Part model, mm, in its own coordinate system. A direction names the side the tool comes from. Give positions to 0.01 mm unless a question says otherwise; leave off trailing zeros. Write each loop counter-clockwise with the first axis right and the second up, starting at its lowest first coordinate (ties: lowest second). Pieces come first, ordered by that corner, then holes. Notation, with made-up numbers: (30, -10) - (57, -10) arc R38 ccw to (57, 28) - close; hole circle Ø3 at (50.25, -7.75). An arc over 180 degrees is marked (long way). Answer as a JSON object with one key per item and string values. Group by question number.
```python
from build123d import *

# Parameters (mm, degrees)
SKETCH_1_R          = 9.15
SKETCH_1_R_2        = 7.15
EXTRUDE_1_DEPTH     = 1
SKETCH_2_W          = 2
SKETCH_2_H          = 11.561648884
CUT_EXTRUDE_1_DEPTH = 13.978636292
EXTRUDE_START       = -1
SKETCH_3_R          = 0.4
EXTRUDE_2_DEPTH     = 1


with BuildPart() as part:
    # 草图1 → 拉伸1 (new body)
    with BuildSketch(Plane(origin=(0, 0, 0), x_dir=(0, 0, -1), z_dir=(1, 0, 0))):
        Circle(SKETCH_1_R)
        Circle(SKETCH_1_R_2, mode=Mode.SUBTRACT)
    extrude(amount=EXTRUDE_1_DEPTH)

    # 草图2 → 切除-拉伸1 (cut, through all)
    with BuildSketch(Plane(origin=(1, 0, 0), x_dir=(0, 0, -1), z_dir=(1, 0, 0))):
        with Locations((0, 5.780824442)):
            Rectangle(SKETCH_2_W, SKETCH_2_H)
    extrude(amount=-CUT_EXTRUDE_1_DEPTH, mode=Mode.SUBTRACT)

    # 草图3 → 拉伸2 (add)
    # profile 1 of 2: a face of its own
    with BuildSketch(Plane(origin=(1, 0, 0), x_dir=(0, 0, -1), z_dir=(1, 0, 0)).offset(EXTRUDE_START)):
        with BuildLine():
            Line((-1, 9.095191037), (-1, 10.12554219))
            Line((-1, 10.12554219), (-2.197020967, 10.125546621))
            ThreePointArc((-2.197020967, 10.125546621), (-2.744657845, 9.962265155), (-3.113455807, 9.525739038))
            Line((-3.113455807, 9.525739038), (-3.599741921, 8.412155378))
            ThreePointArc((-3.599741921, 8.412155378), (-2.325089431, 8.849658702), (-1, 9.095191037))
        make_face()
        with Locations((-2.0521454, 9.383212306)):
            Circle(SKETCH_3_R, mode=Mode.SUBTRACT)
    # profile 2 of 2: a face of its own
    with BuildSketch(Plane(origin=(1, 0, 0), x_dir=(0, 0, -1), z_dir=(1, 0, 0)).offset(EXTRUDE_START)):
        with BuildLine():
            Line((1, 9.095191037), (1, 10.12554219))
            Line((1, 10.12554219), (2.197020967, 10.125546621))
            ThreePointArc((2.197020967, 10.125546621), (2.744657845, 9.962265155), (3.113455807, 9.525739038))
            Line((3.113455807, 9.525739038), (3.599741921, 8.412155378))
            ThreePointArc((3.599741921, 8.412155378), (2.325089431, 8.849658702), (1, 9.095191037))
        make_face()
        with Locations(Location((2.0521454, 9.383212306, 0), (0, 0, 180))):
            Circle(SKETCH_3_R, mode=Mode.SUBTRACT)
    extrude(amount=EXTRUDE_2_DEPTH)


solid = part.part
```
1) Which spindle directions (+Z, -Z, +X, -X, +Y, -Y) get a long thin tool onto all of the face, cutting with end or side? Do faces 4 (the flat face through (0.5, 8.6, 1)), 5 (the flat face through (0, -7, 3)). Say none if no direction does.
2) Saw through at B-B (z = 6.25). List the corners of the cut face in (x, y).
3) Saw through at A-A (y = 0). List the corners of the cut face in (x, z).
4) Two-plate mould, pull along Z, no slides. Class faces 1 (the flat face through (0.49, 8.98, -3.35)), 2 (the cylindrical face through (0.493, -7.144, 0.3)), 3 (the cylindrical face through (0.493, -9.143, 0.351)): +Z half, -Z half, draft (parallel to the pull), parting line (faces both ways), or undercut.
5) Drop a flat-ended pin along its axis: P1, Ø5, axis at y = 6.5, z = 5.5, coming from the -X side. Give the stop position or say it passes through.
6) Saw through at D-D (z = 0). List the corners of the cut face in (x, y).
7) Drill centre lines: line 1 along Z through (x, y) = (0.7, -0.25); line 2 along Z through (x, y) = (0.7, 1.5); line 3 along Y through (x, z) = (0.85, -6.25). Where is each one in solid material? Low to high. Write a range as from..to.
8) Saw through at C-C (x = 0.5). List the corners of the cut face in (y, z), and give its area (3 significant figures).
Checks:
{
 "1": {"face 4": "+X, -X, +Y", "face 5": "+Z, -Z, -X, +Y, -Y"},
 "2": {"outline": "(0, -6.68) - (1, -6.68) - (1, -3.47) - (0, -3.47) - close; (0, 3.47) - (1, 3.47) - (1, 6.68) - (0, 6.68) - close"},
 "3": {"outline": "(0, -9.15) - (1, -9.15) - (1, -7.15) - (0, -7.15) - close; (0, 7.15) - (1, 7.15) - (1, 9.15) - (0, 9.15) - close"},
 "4": {"face 1": "-Z half", "face 2": "undercut", "face 3": "parting line"},
 "5": {"P1": "x = 0"},
 "6": {"outline": "(0, -9.15) - (1, -9.15) - (1, -7.15) - (0, -7.15) - close"},
 "7": {"line 1": "-9.15..-7.15, 7.15..9.15", "line 2": "-9.03..-6.99, 6.99..9.03", "line 3": "-6.68..-3.47, 3.47..6.68"},
 "8": {"outline": "(7.08, -1) arc R7.15 cw (long way) to (7.08, 1) - (10.13, 1) - (10.13, 2.2) arc R1 ccw to (9.53, 3.11) - (8.41, 3.6) arc R9.15 ccw (long way) to (8.41, -3.6) - (9.53, -3.11) arc R1 ccw to (10.13, -2.2) - (10.13, -1) - close; hole circle Ø0.8 at (9.38, -2.05); hole circle Ø0.8 at (9.38, 2.05)", "area": "103 mm2"}
}
